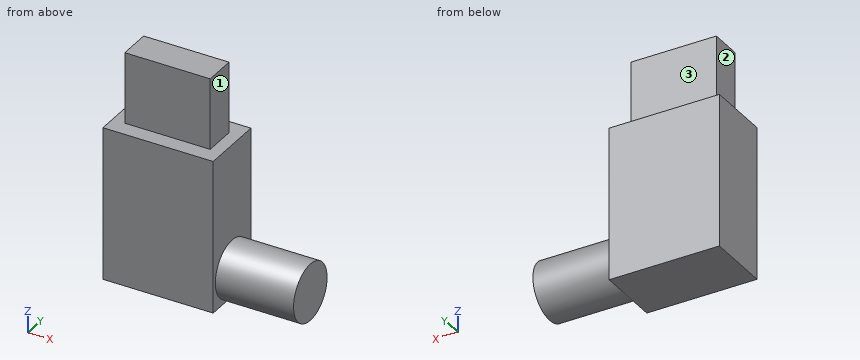
from build123d import *

# Parameters (mm, degrees)
SKETCH_1_W      = 15.5
SKETCH_1_H      = 9
EXTRUDE_1_DEPTH = 21.5
SKETCH_2_R      = 4
EXTRUDE_2_DEPTH = 11
SKETCH_3_W      = 12
SKETCH_3_H      = 4.5
EXTRUDE_3_DEPTH = 10


with BuildPart() as part:
    # 草图1 → 凸台-拉伸1 (new body)
    with BuildSketch(Plane.XY):
        Rectangle(SKETCH_1_W, SKETCH_1_H)
    extrude(amount=-EXTRUDE_1_DEPTH)

    # 草图2 → 凸台-拉伸2 (add)
    with BuildSketch(Plane(origin=(7.75, 0, 0), x_dir=(0, 0, -1), z_dir=(1, 0, 0))):
        with Locations((17.5, 0)):
            Circle(SKETCH_2_R)
    extrude(amount=EXTRUDE_2_DEPTH)

    # 草图3 → 凸台-拉伸3 (add)
    with BuildSketch(Plane.XY):
        Rectangle(SKETCH_3_W, SKETCH_3_H)
    extrude(amount=EXTRUDE_3_DEPTH)


solid = part.part
Part model, mm, in its own coordinate system. Face numbers are marked on the shaded views. A direction names the side the tool comes from. Round coordinates to 2 decimals unless told otherwise and drop trailing zeros. Loops run counter-clockwise (first coordinate to the right, second up) from the corner with the lowest first, then second, coordinate; pieces in that order, holes last. Notation, with made-up numbers: (67.5, 84) - (98.5, 84) arc R24 cw to (98.5, 123) - close; hole circle Ø9 at (42.5, 35). An arc over 180 degrees is marked (long way). Answer as a JSON object with one key per item and string values.
Item 1: Band-saw the part on D-D on z = -4.5. List the corners of the cut face in (x, y), plus the area to 4 significant figures.
Output:
{"outline": "(-7.75, -4.5) - (7.75, -4.5) - (7.75, 4.5) - (-7.75, 4.5) - close", "area": "139.5 mm2"}
Item 2: Band-saw the part on C-C on z = -17.5. List the corners of the cut face in (x, y), plus the area to 4 significant figures.
Output:
{"outline": "(-7.75, -4.5) - (7.75, -4.5) - (7.75, -4) - (18.75, -4) - (18.75, 4) - (7.75, 4) - (7.75, 4.5) - (-7.75, 4.5) - close", "area": "227.5 mm2"}
Item 3: Tool access for the marked faces 1, 2 and 3: list every direction of +Z, -Z, +X, -X, +Y, -Y with a clear straight run to the whole face (end or side of a thin tool).
Output:
{"face 1": "+Z, +X, +Y, -Y", "face 2": "+Z, -X, +Y, -Y", "face 3": "+Z, +X, -X, +Y"}
Item 4: Band-saw the part on B-B on x = -2.5. List the corners of the cut face in (y, z), plus the area to 4 significant figures.
Output:
{"outline": "(-4.5, -21.5) - (4.5, -21.5) - (4.5, 0) - (2.25, 0) - (2.25, 10) - (-2.25, 10) - (-2.25, 0) - (-4.5, 0) - close", "area": "238.5 mm2"}
Item 5: Pin check, flat tips, straight feed: pin 1 (2.5 mm diameter, centred on y = -1.5, z = -11, fed in from +X); pin 2 (1.3 mm diameter, centred on y = -0.5, z = 5.5, fed in from -X); pin 3 (8 mm diameter, centred on x = -0.5, z = 5.5, fed in from -Y). Stop position of each tip, or through.
Output:
{"pin 1": "x = 7.75", "pin 2": "x = -6", "pin 3": "y = -2.25"}
Item 6: Wall check: L1, parallel to Y at x = 1.5, z = 5.5; L2, parallel to X at y = -2.5, z = -13; L3, parallel to Z at x = 4.25, y = 3.25. Give the ranges that are in metal, low to high.
Output:
{"L1": "-2.25 to 2.25", "L2": "-7.75 to 7.75", "L3": "-21.5 to 0"}
